from build123d import *

# Parameters (mm, degrees)
BOSS_EXTRUDE1_DEPTH = 120
CUT_EXTRUDE1_DEPTH  = 55
CUT_EXTRUDE2_DEPTH  = 55
SKETCH5_R           = 10
CUT_EXTRUDE3_DEPTH  = 55
SKETCH6_W           = 70
SKETCH6_H           = 25
BOSS_EXTRUDE2_DEPTH = 120
SKETCH7_R           = 8
CUT_EXTRUDE4_DEPTH  = 25


with BuildPart() as part:
    # Sketch1 → Boss-Extrude1 (new body)
    with BuildSketch(Plane(origin=(0, 0, 0), x_dir=(0, 0, -1), z_dir=(1, 0, 0))):
        Polygon((52, 82.471222814), (52, 17), (0, 17), align=None)
        Polygon((52, 17), (0, 17), (0, 0), (68, 0), (68, 82.471222814), (52, 82.471222814), align=None)
    extrude(amount=-BOSS_EXTRUDE1_DEPTH)

    # Sketch2 → Cut-Extrude1 (cut)
    with BuildSketch(Plane(origin=(0, 0, 0), x_dir=(0, 0, -1), z_dir=(1, 0, 0))):
        Polygon((52, 82.471222814), (0, 17), (52, 17), align=None)
    extrude(amount=-CUT_EXTRUDE1_DEPTH, mode=Mode.SUBTRACT)

    # Sketch3 → Cut-Extrude2 (cut)
    with BuildSketch(Plane.ZY.offset(120)):
        Polygon((-52, 82.471222814), (0, 17), (-52, 17), align=None)
    extrude(amount=-CUT_EXTRUDE2_DEPTH, mode=Mode.SUBTRACT)

    # Sketch5 → Cut-Extrude3 (cut)
    with BuildSketch(Plane.XZ):
        with BuildLine():
            Line((-95, 0), (-120, 0))
            Line((-120, 0), (-120, -25))
            ThreePointArc((-120, -25), (-112.67766953, -7.32233047), (-95, 0))
        make_face()
        with Locations(Location((-95, -25, 0), (0, 0, 270))):
            Circle(SKETCH5_R)
        with BuildLine():
            Line((0, 0), (-25, 0))
            ThreePointArc((-25, 0), (-7.32233047, -7.32233047), (0, -25))
            Line((0, -25), (0, 0))
        make_face()
        with Locations(Location((-25, -25, 0), (0, 0, 270))):
            Circle(SKETCH5_R)
    extrude(amount=-CUT_EXTRUDE3_DEPTH, mode=Mode.SUBTRACT)

    # Sketch6 → Boss-Extrude2 (add)
    with BuildSketch(Plane(origin=(0, 0, 0), x_dir=(0, 0, -1), z_dir=(1, 0, 0))):
        with Locations((103, 69.971222814)):
            Rectangle(SKETCH6_W, SKETCH6_H)
    extrude(amount=-BOSS_EXTRUDE2_DEPTH)

    # Sketch7 → Cut-Extrude4 (cut)
    with BuildSketch(Plane(origin=(0, 82.471222814, 0), x_dir=(1, 0, 0), z_dir=(0, 1, 0))):
        with Locations(Location((-60, 103, 0), (0, 0, 270))):
            Circle(SKETCH7_R)
        with BuildLine():
            Line((0, 138), (-60, 138))
            ThreePointArc((-60, 138), (-42.081937118, 133.065645221), (-29.216107334, 119.653887004))
            Line((-29.216107334, 119.653887004), (0, 65.649346677))
            Line((0, 65.649346677), (0, 138))
        make_face()
        with BuildLine():
            Line((-120, 138), (-120, 65.649346677))
            Line((-120, 65.649346677), (-90.783892666, 119.653887004))
            ThreePointArc((-90.783892666, 119.653887004), (-77.918062882, 133.065645221), (-60, 138))
            Line((-60, 138), (-120, 138))
        make_face()
    extrude(amount=-CUT_EXTRUDE4_DEPTH, mode=Mode.SUBTRACT)


solid = part.part
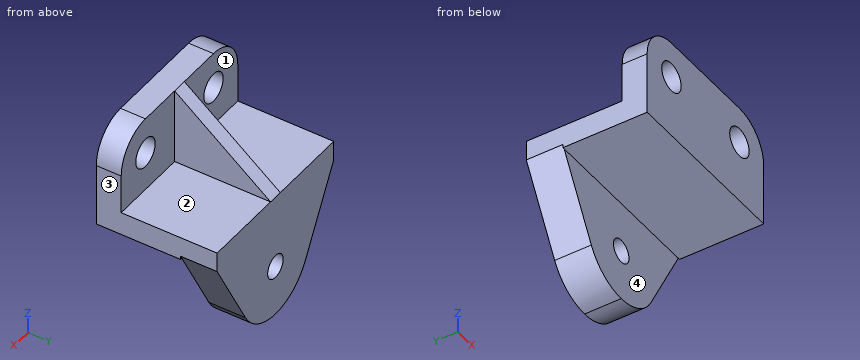
The listing builds one solid part. Answer for the finished solid, in the listing's coordinates (mm). Face numbers are marked on the shaded views. A direction names the side the tool comes from. Coordinates: 2 decimals unless noted, no trailing zeros. Write each loop counter-clockwise with the first axis right and the second up, starting at its lowest first coordinate (ties: lowest second). Pieces come first, ordered by that corner, then holes. Notation, with made-up numbers: M 77.25,38.5 L 131.25,38.5 A26 ccw 131.25,67.5 Z; hole C 32.25,-12 d3. An arc over 180 degrees is marked long. Put each result on its own line as item: value. Start each with the question number.
1. Consider line 1 (X direction, y = 10.75, z = -25); line 2 (Y direction, x = -34.5, z = -97.5); line 3 (Z direction, x = -98.5, y = 35.5). Determine where each line is inside the solid, lowest interval first. Write a range as from..to.
2. A cutting plane is placed at D-D on x = -108. Write down the section's boundary in (y, z).
3. A cutting plane is placed at B-B on y = 69. Write down the section's boundary in (x, z).
4. A cutting plane is placed at A-A on z = -33. Write down the section's boundary in (x, y).
5. A cutting plane is placed at C-C on z = -103. Write down the section's boundary in (x, y), then the cut area to 3 significant figures.
6. Flat-ended cylindrical pins translate along their axes: P1, Ø3, axis at x = -20, z = -32.5, coming from the +Y side; P2, Ø16.5, axis at x = -25, y = 61.5, coming from the +Z side; P3, Ø6, axis at y = 56, z = -28.5, coming from the -X side. Find the tip coordinate at first contact, or state that the pin passes through.
7. Which of the six approach directions +Z, -Z, +X, -X, +Y, -Y give full straight-line access (tool end or side, diameter ignored) to the marked faces 1, 2, 3 and 4?
Resolved:
1. line 1: x = -120..-105, -85..-35, -15..0
1. line 2: y = 57.47..82.47
1. line 3: z = -68..-52
2. outline: M 0,-68 L 57.47,-68 L 57.47,-87.83 L 82.47,-87.83 L 82.47,-52 L 17,-52 L 17,-3.65 L 0,-3.65 Z
3. outline: M -120,-65.65 L -90.78,-119.65 A35 ccw -29.22,-119.65 L 0,-65.65 L 0,-52 L -55,-52 L -55,-41.3 L -65,-41.3 L -65,-52 L -120,-52 Z; hole C -60,-103 d16
4. outline: M -120,0 L -101,0 L -101,17 L -120,17 Z; M -89,0 L -31,0 L -31,17 L -55,17 L -55,58.55 L -65,58.55 L -65,17 L -89,17 Z; M -19,0 L 0,0 L 0,17 L -19,17 Z
5. outline: M -99.79,57.47 L -68,57.47 L -68,82.47 L -99.79,82.47 Z; M -52,57.47 L -20.21,57.47 L -20.21,82.47 L -52,82.47 Z
5. area: 1,590 mm2
6. P1: stops at y = 17
6. P2: stops at z = -52
6. P3: stops at x = -65
7. face 1: +Z, -X, +Y
7. face 2: +Z, +X, +Y
7. face 3: +Z, -Z, +X, +Y, -Y
7. face 4: -Z, +X, -X, -Y
